Geometry: final body of the model. Coordinates: model frame, mm. A direction names the side the tool comes from. Round coordinates to 2 decimals unless told otherwise and drop trailing zeros. Write each loop counter-clockwise with the first axis right and the second up, starting at its lowest first coordinate (ties: lowest second). Pieces come first, ordered by that corner, then holes. Notation, with made-up numbers: M -32,8.25 L 20,8.25 A19 ccw 20,27.25 Z; hole C -35.75,-16 d8. An arc over 180 degrees is marked long. Use one line per item in the form item = value. Start each with the question number.
from build123d import *

# Parameters (mm, degrees)
TRACK_PROFILE_SKETCH_W            = 30
TRACK_PROFILE_SKETCH_H            = 10
TRACK_BODY_200MM_DEPTH            = 100
EDGE_CHAMFER_5MM_SIZE             = 5
GUIDE_GROOVE_SKETCH_W             = 10
GUIDE_GROOVE_SKETCH_H             = 200
GUIDE_GROOVE_10X5_DEPTH           = 5
END_START                         = -200
END_NOTCH_SKETCH_W                = 15
END_NOTCH_SKETCH_H                = 1.5
END_NOTCH_CUT_DEPTH               = 200
RACK_POCKET_CUT_REACH             = 103.242
RACK_POCKET_SKETCH_W              = 5
RACK_POCKET_SKETCH_H              = 5
RACK_POCKET_PATTERN_20X10MM_COUNT = 20
RACK_POCKET_PATTERN_20X10MM_PITCH = 10


with BuildPart() as part:
    # Track Profile Sketch → Track Body 200mm (new, symmetric)
    with BuildSketch(Plane.XY):
        Rectangle(TRACK_PROFILE_SKETCH_W, TRACK_PROFILE_SKETCH_H)
    extrude(amount=TRACK_BODY_200MM_DEPTH, both=True)

    # Edge Chamfer 5mm
    edge_chamfer_5mm_edges = [part.edges().sort_by_distance(p)[0] for p in [
        (-15, 5, 0),
        (15, 5, 0),
    ]]
    chamfer(edge_chamfer_5mm_edges, length=EDGE_CHAMFER_5MM_SIZE)

    # Guide Groove Sketch → Guide Groove 10x5 (cut)
    with BuildSketch(Plane(origin=(0, 5, 0), x_dir=(1, 0, 0), z_dir=(0, 1, 0))):
        Rectangle(GUIDE_GROOVE_SKETCH_W, GUIDE_GROOVE_SKETCH_H)
    extrude(amount=-GUIDE_GROOVE_10X5_DEPTH, mode=Mode.SUBTRACT)

    # End Notch Sketch → End Notch Cut (cut)
    with BuildSketch(Plane.XY.offset(100).offset(END_START)):
        with Locations((0, 0.75)):
            Rectangle(END_NOTCH_SKETCH_W, END_NOTCH_SKETCH_H)
    extrude(amount=END_NOTCH_CUT_DEPTH, mode=Mode.SUBTRACT)

    # Rack Pocket Sketch → Rack Pocket Cut (cut, up to next)
    with BuildSketch(Plane(origin=(0, 0, 0), x_dir=(1, 0, 0), z_dir=(0, 1, 0)), mode=Mode.PRIVATE) as rack_pocket_cut_sk1:
        with Locations((0, 95.5)):
            Rectangle(RACK_POCKET_SKETCH_W, RACK_POCKET_SKETCH_H)
    rack_pocket_cut_tool1 = extrude(rack_pocket_cut_sk1.sketch, amount=-RACK_POCKET_CUT_REACH, mode=Mode.PRIVATE) & part.part
    rack_pocket_cut = rack_pocket_cut_tool1.solids().sort_by_distance((0, 0, -95.5))[0]
    add(rack_pocket_cut, mode=Mode.SUBTRACT)

    # Rack Pocket Pattern 20x10mm: Rack Pocket Cut ×20
    with Locations(*[(0, 0, i * RACK_POCKET_PATTERN_20X10MM_PITCH) for i in range(1, RACK_POCKET_PATTERN_20X10MM_COUNT)]):
        add(rack_pocket_cut, mode=Mode.SUBTRACT)


solid = part.part
1. Section query A-A (z = -10.5). Return loops of the section in (x, y), then the cut area to 4 significant figures.
2. Pull-direction query (X, two-part tool) for faces 1 (the face through (0, -1, 100)), 2 (the face through (2.5, -2, 55)); classes: released by +X, released by -X, zero draft, split by the parting line, or undercut.
3. Ray query, probe 1 along X at (y, z) = (-2.75, 73); probe 2 along Y at (x, z) = (-3, 68); probe 3 along X at (y, z) = (3, -24). Return the intervals inside material, ascending.
4. Set-up query: faces 3 (the face through (-8, 5, 1)), 4 (the face through (0, -2, -13)), 5 (the face through (-5, 3, 1)). Return all of +Z, -Z, +X, -X, +Y, -Y with unobstructed straight access to the full face (end or side cutting, diameter ignored); none if empty.
5. Section query B-B (x = 12.5). Return loops of the section in (y, z).
6. Contact query for flat-ended pins moving along their axis: pin 1 (1.5 mm diameter, centred on x = -2, z = 25, fed in from +Y); pin 2 (1.6 mm diameter, centred on y = 1, z = -49, fed in from -X). Output: stop coordinate, or through.
Checks:
q1.outline = M -15,-5 L 15,-5 L 15,0 L 10,5 L 5,5 L 5,1.5 L 7.5,1.5 L 7.5,0 L -7.5,0 L -7.5,1.5 L -5,1.5 L -5,5 L -10,5 L -15,0 Z
q1.area = 217.5 mm^2
q2.face_1 = zero draft
q2.face_2 = undercut
q3.probe_1 = -15 to -2.5, 2.5 to 15
q3.probe_2 = -5 to 0
q3.probe_3 = -12 to -5, 5 to 12
q4.face_3 = +Z, -Z, +X, -X, +Y
q4.face_4 = +Y, -Y
q4.face_5 = +Z, -Z, +Y
q5.outline = M -5,-100 L 2.5,-100 L 2.5,100 L -5,100 Z
q6.pin_1 = 0
q6.pin_2 = -14.8
